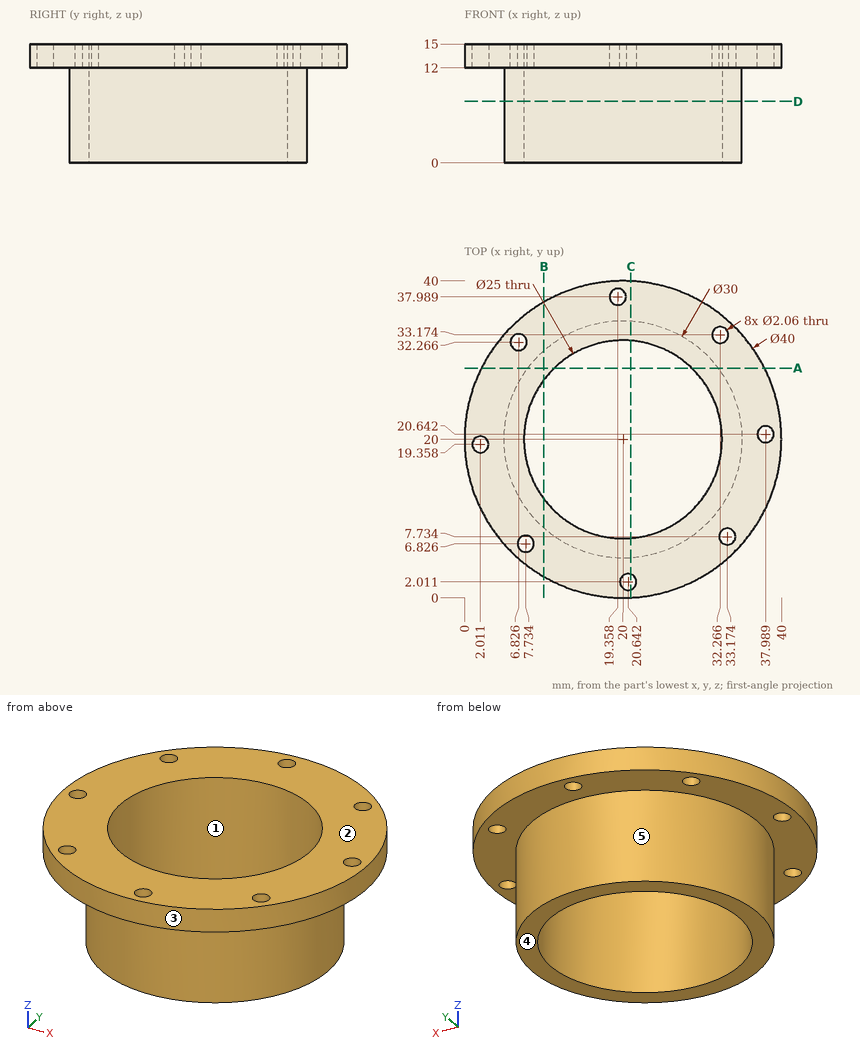
Check sheet for the drawn part. Datum: minimum x, y, z corner. Units: mm. A direction names the side the tool comes from. Round coordinates to 2 decimals unless told otherwise and drop trailing zeros. Loops run counter-clockwise (first coordinate to the right, second up) from the corner with the lowest first, then second, coordinate; pieces in that order, holes last. Notation, with made-up numbers: (-37, -25) -> (-16, -25) arc R20 ccw to (-16, -10) -> close; hole circle Ø5 at (52.5, 86.25). An arc over 180 degrees is marked (long way). Put each result on its own line as item: value. Start each with the question number.
1. Section check C-C (x = 21). Enter the section's corners in (y, z) (1 decimal).
2. Gauge pin test, flat ends, axial feed: pin 1 (5 mm diameter, centred on y = 5, z = 5.5, fed in from +X); pin 2 (3.5 mm diameter, centred on x = 7.73, y = 6.83, fed in from -Z); pin 3 (5 mm diameter, centred on x = 22, z = 3.5, fed in from -Y). Record the tip position at first contact, or that the pin passes through.
3. Section check B-B (x = 10). Enter the section's corners in (y, z).
4. Access from +Z, -Z, +X, -X, +Y, -Y to the whole of each face (thin tool, end or side, straight path). Record for the marked faces 4 and 5.
5. Draft check along Y on the marked faces 1, 2 and 3. Enter one of: +Y half, -Y half, draft (parallel to the pull), parting line (faces both ways), or undercut.
6. Section check A-A (y = 29). Enter the section's corners in (x, z) (1 decimal).
7. Section check D-D (z = 7.75). Enter the section's corners in (x, y).
8. Scan lines: probe 1 along Z at (x, y) = (10.5, 8); probe 2 along Y at (x, z) = (12, 9.75) (1 decimal); probe 3 along X at (y, z) = (9, 0.5) (1 decimal). Record each from-to range of solid material in increasing order.
Findings:
1. outline: (0, 12) -> (1, 12) -> (1, 15) -> (0, 15) -> close; (3, 12) -> (5, 12) -> (5, 0) -> (7.5, 0) -> (7.5, 15) -> (3, 15) -> close; (32.5, 0) -> (35, 0) -> (35, 12) -> (40, 12) -> (40, 15) -> (32.5, 15) -> close
2. pin 1: stops at x = 28.29
2. pin 2: stops at z = 12
2. pin 3: stops at y = 5
3. outline: (2.68, 12) -> (8.82, 12) -> (8.82, 0) -> (12.5, 0) -> (12.5, 15) -> (2.68, 15) -> close; (27.5, 0) -> (31.18, 0) -> (31.18, 12) -> (37.32, 12) -> (37.32, 15) -> (27.5, 15) -> close
4. face 4: -Z, +X, -X, +Y, -Y
4. face 5: -Z
5. face 1: undercut
5. face 2: draft
5. face 3: parting line
6. outline: (2.1, 12) -> (8, 12) -> (8, 0) -> (11.3, 0) -> (11.3, 15) -> (2.1, 15) -> close; (28.7, 0) -> (32, 0) -> (32, 12) -> (37.9, 12) -> (37.9, 15) -> (28.7, 15) -> close
7. outline: circle Ø30 at (20, 20); hole circle Ø25 at (20, 20)
8. probe 1: z = 12 to 15
8. probe 2: y = 7.3 to 10.4, 29.6 to 32.7
8. probe 3: x = 9.8 to 14.1, 25.9 to 30.2
